Study the drawing (mm; zero at the part's minimum x, y, z) and answer. Round coordinates to 2 decimals unless told otherwise and drop trailing zeros. Write each loop counter-clockwise with the first axis right and the second up, starting at its lowest first coordinate (ties: lowest second). Pieces come first, ordered by that corner, then holes.
(1) A cutting plane is placed at A-A, the plane y = 4. Give the vertices of the cut face in (x, z), and give its area (3 significant figures).
(2) Find the intervals of material crossed by probe 1 along X at (y, z) = (7, 6.75) (1 decimal); probe 2 along Z at (x, y) = (11.75, 7); probe 3 along Z at (x, y) = (11.5, 4.25), in increasing order.
(3) The mould has two halves that part along X. Classify the marked faces 1, 2, 3 and 4: +X half, -X half, draft (parallel to the pull), parting line (faces both ways), or undercut.
(4) Each of these flat-tipped pins is pushed along its axis until it touches: pin 1 Ø1.5 at (x, z) = (2.5, 9) entering from -Y; pin 2 Ø1 at (x, z) = (12, 8.5) entering from +Y. Where does it stop, or does it pass through?
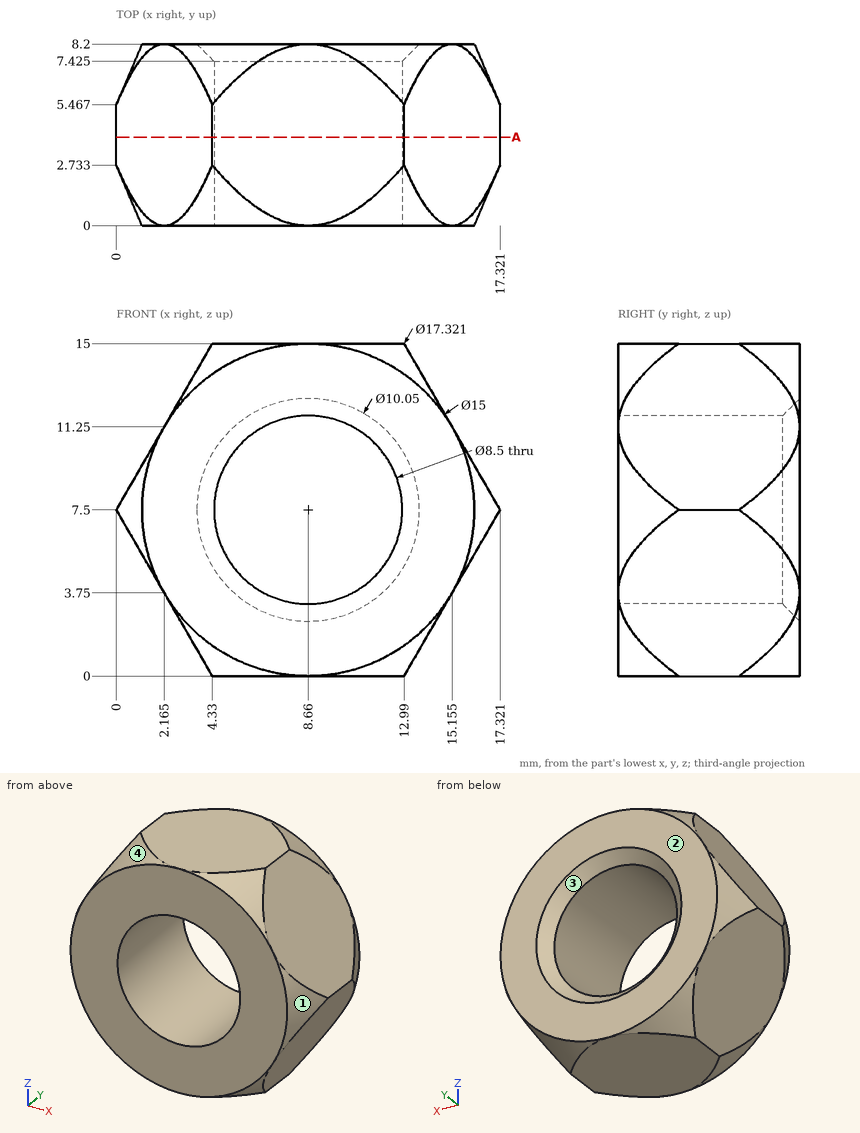
Solutions:
1. outline: (0, 7.5) - (4.33, 0) - (12.99, 0) - (17.32, 7.5) - (12.99, 15) - (4.33, 15) - close; hole circle Ø8.5 at (8.66, 7.5)
1. area: 138 mm2
2. probe 1: x = 0.7 to 4.5, 12.8 to 16.6
2. probe 2: z = 0.11 to 4.58, 10.42 to 14.89
2. probe 3: z = 0 to 4.34, 10.66 to 15
3. face 1: +X half
3. face 2: draft
3. face 3: undercut
3. face 4: -X half
4. pin 1: stops at y = 0
4. pin 2: passes through
